For this review, take the finished solid that the model builds, in its own axes (mm). Round coordinates to 2 decimals unless told otherwise and drop trailing zeros. Loops run counter-clockwise (first coordinate to the right, second up) from the corner with the lowest first, then second, coordinate; pieces in that order, holes last.
1) Insertion check: pin 1 (5.5 mm diameter, centred on x = 0, y = 0, fed in from -Z); pin 2 (5 mm diameter, centred on x = 35, z = 3.5, fed in from +Y); pin 3 (2 mm diameter, centred on x = 38.5, y = 114, fed in from -Z); pin 4 (2 mm diameter, centred on y = 76.5, z = 6.5, fed in from -X). Each pin has a flat end and moves straight along its axis. Give the tip position at first contact, or say it passes through.
2) Take a section at D-D (y = 193.5). State the section outline as (x, z) points, then the cut area to 3 significant figures.
3) Take a section at A-A (y = 124.5). State the section outline as (x, z) points.
4) Wall thickness on L1, parallel to Y at x = 0, z = 7.5; L2, parallel to X at y = 99.5, z = 1.25; L3, parallel to X at y = 97.5, z = 6.25: over which ranges is each line inside the solid? List them lowest first.
5) Take a section at C-C (x = 54.5). State the section outline as (y, z) points.
6) Take a section at B-B (z = 8). Give the number of separate pieces and of enclosed holes in the cut face, then the cut area to 3 significant figures.
```python
from build123d import *

# Parameters (mm, degrees)
SKETCH_1_R      = 3
SKETCH_1_R_2    = 16
SKETCH_1_R_3    = 3.91899873
SKETCH_1_R_4    = 2
EXTRUDE_1_DEPTH = 10


with BuildPart() as part:
    # 草图1 → 凸台-拉伸1 (new body)
    with BuildSketch(Plane.XY):
        with BuildLine():
            Line((-14, 112), (-6, 0))
            ThreePointArc((-6, 0), (0, -6), (6, 0))
            add(Edge.make_bspline(
                [(6, 0), (1.588652615, 45.680929706), (5.604102499, 63.643200211), (28.004797731, 96.13093391)],
                knots=[0, 0, 0, 0, 0.788155359, 0.788155359, 0.788155359, 0.788155359], degree=3))
            ThreePointArc((28.004797731, 96.13093391), (50.113637924, 112.900750568), (77, 119.767416406))
            ThreePointArc((77, 119.767416406), (157.787149523, 154.485384951), (196.379869136, 233.494896157))
            ThreePointArc((196.379869136, 233.494896157), (200.439238403, 236.311917913), (202, 241))
            Line((202, 241), (202, 246))
            ThreePointArc((202, 246), (194.5, 253.5), (187, 246))
            ThreePointArc((187, 246), (154.781745931, 168.218254069), (77, 136))
            Line((77, 136), (10, 136))
            ThreePointArc((10, 136), (-6.970562748, 128.970562748), (-14, 112))
        make_face()
        Circle(SKETCH_1_R, mode=Mode.SUBTRACT)
        with Locations((10, 112)):
            Circle(SKETCH_1_R_2, mode=Mode.SUBTRACT)
        with Locations((194.5, 246)):
            Circle(SKETCH_1_R_3, mode=Mode.SUBTRACT)
        with Locations((0, 12.5)):
            Circle(SKETCH_1_R_4, mode=Mode.SUBTRACT)
    extrude(amount=EXTRUDE_1_DEPTH)


solid = part.part
```
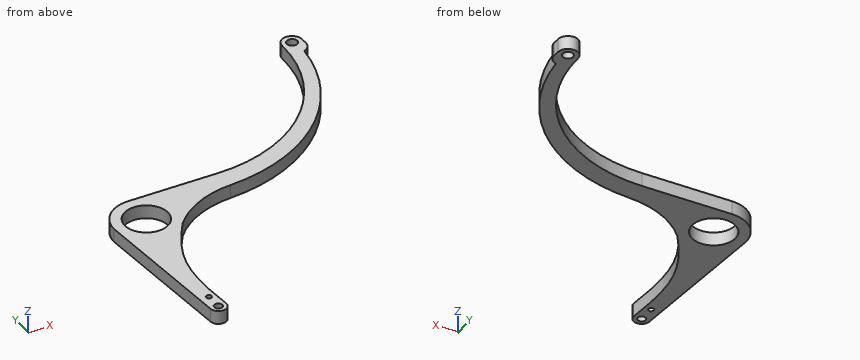
Response:
1. pin 1: passes through
1. pin 2: stops at y = 136
1. pin 3: stops at z = 0
1. pin 4: stops at x = -11.54
2. outline: (173.66, 0) - (185.58, 0) - (185.58, 10) - (173.66, 10) - close
2. area: 119 mm2
3. outline: (-10.49, 0) - (0.01, 0) - (0.01, 10) - (-10.49, 10) - close; (19.99, 0) - (105.44, 0) - (105.44, 10) - (19.99, 10) - close
4. L1: y = -6 to -3, 3 to 10.5, 14.5 to 99.51, 124.49 to 133.82
4. L2: x = -13.11 to 0.01, 19.99 to 31.18
4. L3: x = -12.96 to 3.24, 16.76 to 29.24
5. outline: (114.83, 0) - (136, 0) - (136, 10) - (114.83, 10) - close
6. separate pieces: 1
6. enclosed holes: 4
6. area: 6,110 mm2
